Could you check a few things on this drawing? It's one solid part, dimensions in mm from its lowest x, y, z. Round coordinates to 2 decimals unless told otherwise and drop trailing zeros. Write each loop counter-clockwise with the first axis right and the second up, starting at its lowest first coordinate (ties: lowest second). Pieces come first, ordered by that corner, then holes. Notation, with made-up numbers: M -34,26 L 4,26 A19 ccw 4,51 Z; hole C 47.25,88 d3. An arc over 180 degrees is marked long. One line per question, with ' | ' between items. Start each with the question number.
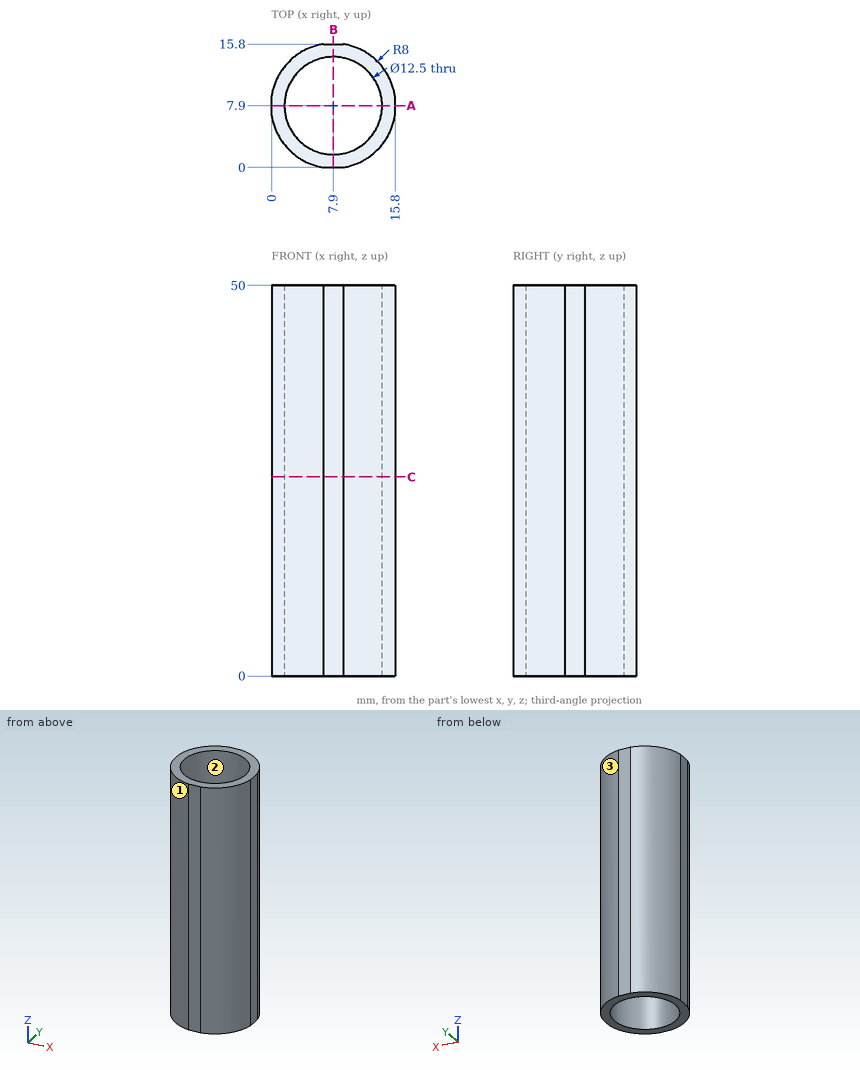
1. Suppose I cut it at C-C (z = 25.5). Write out the boundary of the cut face in (x, y).
2. If we mould it in two halves opening along X, with no side actions, what happens to the marked faces 1, 2 and 3? For each: released by +X, released by -X, zero draft, split by the parting line, or undercut.
3. I'm going to push flat-ended pins straight in: P1, Ø3, axis at x = 3.5, y = 11.5, coming from the -Z side; P2, Ø1.5, axis at x = 4.5, z = 24, coming from the -Y side; P3, Ø2, axis at x = 9, y = 11, coming from the -Z side. Where does each tip first touch, or does it pass through?
4. I need wall thicknesses on line 1 along Y through (x, z) = (7.9, 23.5); line 2 along Y through (x, z) = (12.25, 39.5); line 3 along X through (y, z) = (5.25, 11.5). Which ranges of each line are inside material? Lowest first, please. Write a range as from..to.
5. Suppose I cut it at A-A (y = 7.9). Write out the boundary of the cut face in (x, z), and give its area (3 significant figures).
Computed:
1) outline: M 0,6.64 A8 ccw 6.64,0 L 9.16,0 A8 ccw 15.8,6.64 L 15.8,9.16 A8 ccw 9.16,15.8 L 6.64,15.8 A8 ccw 0,9.16 Z; hole C 7.9,7.9 d12.5
2) face 1: released by -X | face 2: undercut | face 3: released by +X
3) P1: stops at z = 0 | P2: stops at y = 0.35 | P3: passes through
4) line 1: y = 0..1.65, 14.15..15.8 | line 2: y = 1.19..3.41, 12.39..14.61 | line 3: x = 0.35..2.24, 13.56..15.45
5) outline: M 0,0 L 1.65,0 L 1.65,50 L 0,50 Z; M 14.15,0 L 15.8,0 L 15.8,50 L 14.15,50 Z | area: 165 mm²
